from build123d import *

# Parameters (mm, degrees)
CENTER_BODY_SKETCH_W         = 80
CENTER_BODY_SKETCH_H         = 64
CENTER_BODY_SKETCH_R         = 17.5
CENTER_BODY_DEPTH            = 44
PIVOT_EYES_SKETCH_R          = 34
PIVOT_EYES_SKETCH_R_2        = 23.5
PIVOT_EYES_68X_47_DEPTH      = 15.75
PIVOT_EYES_68X_47_2_DEPTH    = 15.75
EYE_FACE_PADS_SKETCH_R       = 34
EYE_FACE_PADS_SKETCH_R_2     = 23.5
EYE_FACE_PADS_DEPTH          = 1.25
MOUNTING_LUG_A_SKETCH_W      = 27.466221721
MOUNTING_LUG_A_SKETCH_H      = 44
MOUNTING_LUG_A_SKETCH_R      = 4
MOUNTING_LUG_A_DEPTH         = 7
MOUNTING_START               = -14
MOUNTING_LUG_B_SKETCH_R      = 4
MOUNTING_LUG_B_DEPTH         = 14
OFFSET_PIVOT_EYES_SKETCH_R   = 34
OFFSET_PIVOT_EYES_SKETCH_R_2 = 23.5
OFFSET_PIVOT_EYES_DEPTH      = 8.5
CENTER_WEB_SKETCH_W          = 28.251394121
CENTER_WEB_SKETCH_H          = 44
CENTER_WEB_DEPTH             = 14
PIN_HOLE_SKETCH_R            = 3.5
PIN_HOLE_7_DEPTH             = 200
LUG_A_FILLETS_R5_R           = 5
LUG_B_FILLETS_R5_R           = 5


with BuildPart() as part:
    # Center Body Sketch → Center Body (new body)
    with BuildSketch(Plane(origin=(0, 0, 0), x_dir=(1, 0, 0), z_dir=(0, 1, 0))):
        Rectangle(CENTER_BODY_SKETCH_W, CENTER_BODY_SKETCH_H)
        with Locations(Location((0, 0, 0), (0, 0, 270))):
            Circle(CENTER_BODY_SKETCH_R, mode=Mode.SUBTRACT)
    extrude(amount=CENTER_BODY_DEPTH)



with BuildPart() as body_2:
    # Pivot Eyes Sketch → Pivot Eyes Ø68xØ47 (new body)
    with BuildSketch(Plane.XY.offset(32)):
        with Locations((-92.2, 22)):
            Circle(PIVOT_EYES_SKETCH_R)
        with Locations((-92.2, 22)):
            Circle(PIVOT_EYES_SKETCH_R_2, mode=Mode.SUBTRACT)
    extrude(amount=-PIVOT_EYES_68X_47_DEPTH)



with BuildPart() as body_3:
    # Pivot Eyes Sketch → Pivot Eyes _68x_47 2 (new body)
    with BuildSketch(Plane.XY.offset(32)):
        with Locations((92.2, 22)):
            Circle(PIVOT_EYES_SKETCH_R)
        with Locations((92.2, 22)):
            Circle(PIVOT_EYES_SKETCH_R_2, mode=Mode.SUBTRACT)
    extrude(amount=-PIVOT_EYES_68X_47_2_DEPTH)


with BuildPart() as body_2_1:
    add(body_2.part)

    add(body_3.part)  # Eye Face Pads merges body 3
    # Eye Face Pads Sketch → Eye Face Pads (add)
    # profile 1 of 2: a face of its own
    with BuildSketch(Plane.XY.offset(32)):
        with Locations((-92.2, 22)):
            Circle(EYE_FACE_PADS_SKETCH_R)
        with Locations((-92.2, 22)):
            Circle(EYE_FACE_PADS_SKETCH_R_2, mode=Mode.SUBTRACT)
    # profile 2 of 2: a face of its own
    with BuildSketch(Plane.XY.offset(32)):
        with Locations((92.2, 22)):
            Circle(EYE_FACE_PADS_SKETCH_R)
        with Locations((92.2, 22)):
            Circle(EYE_FACE_PADS_SKETCH_R_2, mode=Mode.SUBTRACT)
    extrude(amount=EYE_FACE_PADS_DEPTH)


with BuildPart() as part_1:
    add(part.part)

    add(body_2_1.part)  # Mounting Lug A merges body 2
    # Mounting Lug A Sketch → Mounting Lug A (add, symmetric)
    # profile 1 of 2: a face of its own
    with BuildSketch(Plane.XY.offset(25)):
        with Locations((53.733110861, 22)):
            Rectangle(MOUNTING_LUG_A_SKETCH_W, MOUNTING_LUG_A_SKETCH_H)
    # profile 2 of 2: a face of its own
    with BuildSketch(Plane.XY.offset(25)):
        with BuildLine():
            Line((-40, 44), (-40, 0))
            Line((-40, 0), (-66.277037206, 0))
            ThreePointArc((-66.277037206, 0), (-61.345502759, 36.282856857), (-92.2, 56))
            ThreePointArc((-92.2, 56), (-89.821719025, 56.601843613), (-88.015979336, 58.262488159))
            Line((-88.015979336, 58.262488159), (-73.833659926, 79.93878434))
            ThreePointArc((-73.833659926, 79.93878434), (-60.894229811, 86.47759422), (-48.760320341, 78.543293537))
            Line((-48.760320341, 78.543293537), (-32.680005104, 46.743691884))
            ThreePointArc((-32.680005104, 46.743691884), (-30.837059719, 44.740801685), (-28.218046601, 44))
            Line((-28.218046601, 44), (-40, 44))
        make_face()
        with Locations((-61.7, 72)):
            Circle(MOUNTING_LUG_A_SKETCH_R, mode=Mode.SUBTRACT)
    extrude(amount=MOUNTING_LUG_A_DEPTH, both=True)

    # Mounting Lug B Sketch → Mounting Lug B (add)
    with BuildSketch(Plane(origin=(0, 0, -32), x_dir=(-1, 0, 0), z_dir=(0, 0, -1)).offset(MOUNTING_START)):
        with BuildLine():
            Line((-40, 44), (-25.135268802, 44))
            ThreePointArc((-25.135268802, 44), (-27.59760019, 44.648342369), (-29.421358071, 46.425230346))
            Line((-29.421358071, 46.425230346), (-49.270341118, 79.466831997))
            ThreePointArc((-49.270341118, 79.466831997), (-61.764908832, 86.499854718), (-74.196010179, 79.355251839))
            Line((-74.196010179, 79.355251839), (-86.507393015, 58.439154252))
            ThreePointArc((-86.507393015, 58.439154252), (-88.41197553, 56.591508495), (-90.993751524, 55.978595683))
            ThreePointArc((-90.993751524, 55.978595683), (-61.096956424, 35.733196289), (-66.277037206, 0))
            Line((-66.277037206, 0), (-40, 0))
            Line((-40, 0), (-40, 44))
        make_face()
        with Locations((-61.7, 72)):
            Circle(MOUNTING_LUG_B_SKETCH_R, mode=Mode.SUBTRACT)
    extrude(amount=MOUNTING_LUG_B_DEPTH)

    # Offset Pivot Eyes Sketch → Offset Pivot Eyes (add, symmetric)
    # profile 1 of 2: a face of its own
    with BuildSketch(Plane.XY.offset(-25)):
        with Locations((92.2, 22)):
            Circle(OFFSET_PIVOT_EYES_SKETCH_R)
        with Locations((92.2, 22)):
            Circle(OFFSET_PIVOT_EYES_SKETCH_R_2, mode=Mode.SUBTRACT)
    # profile 2 of 2: a face of its own
    with BuildSketch(Plane.XY.offset(-25)):
        with Locations((-92.2, 22)):
            Circle(OFFSET_PIVOT_EYES_SKETCH_R)
        with Locations((-92.2, 22)):
            Circle(OFFSET_PIVOT_EYES_SKETCH_R_2, mode=Mode.SUBTRACT)
    extrude(amount=OFFSET_PIVOT_EYES_DEPTH, both=True)


with BuildPart() as offset_pivot_eyes_piece_1:
    # of the separate pieces the step leaves, piece 1, a body of its own (offset_pivot_eyes_pieces)
    add(part_1.part.solids().sort_by_distance((126.2, 22, -33.5))[0])



with BuildPart() as offset_pivot_eyes_piece_2:
    # of the separate pieces the step leaves, piece 2, a body of its own (offset_pivot_eyes_pieces)
    add(part_1.part.solids().sort_by_distance((-58.2, 22, -33.5))[0])


with BuildPart() as offset_pivot_eyes_piece_1_1:
    add(offset_pivot_eyes_piece_1.part)

    add(offset_pivot_eyes_piece_2.part)  # Center Web merges Offset Pivot Eyes piece 2
    # Center Web Sketch → Center Web (add)
    with BuildSketch(Plane(origin=(0, 0, -32), x_dir=(-1, 0, 0), z_dir=(0, 0, -1))):
        with Locations((54.125697061, 22)):
            Rectangle(CENTER_WEB_SKETCH_W, CENTER_WEB_SKETCH_H)
    extrude(amount=-CENTER_WEB_DEPTH)

    # Pin Hole Sketch → Pin Hole Ø7 (cut)
    with BuildSketch(Plane(origin=(0, 0, -32), x_dir=(-1, 0, 0), z_dir=(0, 0, -1))):
        with Locations((0, 22)):
            Circle(PIN_HOLE_SKETCH_R)
    extrude(amount=-PIN_HOLE_7_DEPTH, mode=Mode.SUBTRACT)

    # Lug A Fillets R5
    lug_a_fillets_r5_edges = [offset_pivot_eyes_piece_1_1.edges().sort_by_distance(p)[0] for p in [
        (-40, 22, -18),
        (-40, 22, 18),
    ]]
    fillet(lug_a_fillets_r5_edges, radius=LUG_A_FILLETS_R5_R)

    # Lug B Fillets R5
    lug_b_fillets_r5_edges = [offset_pivot_eyes_piece_1_1.edges().sort_by_distance(p)[0] for p in [
        (40, 22, 18),
        (40, 22, -18),
    ]]
    fillet(lug_b_fillets_r5_edges, radius=LUG_B_FILLETS_R5_R)


solid = offset_pivot_eyes_piece_1_1.part
Design review of the part built by this model. Coordinates are the model's own, in mm. A direction names the side the tool comes from. Round coordinates to 2 decimals unless told otherwise and drop trailing zeros. Write each loop counter-clockwise with the first axis right and the second up, starting at its lowest first coordinate (ties: lowest second). Pieces come first, ordered by that corner, then holes. Notation, with made-up numbers: M -38,-30.5 L -13,-30.5 A18 cw -13,-16.5 Z; hole C 74,52 d11. An arc over 180 degrees is marked long. One line per item, written item: value. Start each with the question number.
1. Clearance check with flat-ended pins moving along their axes: P1, Ø1, axis at x = 30, y = 16, coming from the +Z side; P2, Ø6, axis at y = 8.5, z = 5.5, coming from the +X side; P3, Ø3, axis at x = -50, z = 22.5, coming from the +Y side. State where each tip first meets the part, or that it passes through.
2. Take a section at B-B on z = 24. State the section outline as (x, y) points.
3. Take a section at C-C on y = 61.5. State the section outline as (x, z) points, then the cut area to 3 significant figures.
4. Take a section at D-D on z = 0. State the section outline as (x, y) points.
5. Draft analysis for pull direction Z (two halves, no side actions). For faces 6 (the face through (5.26, 21.69, 16.69)), 7 (the face through (27.566, 44.631, -24.902)), 8 (the face through (-115, 15, -33.5)), state which applies: pulls with the +Z half, pulls with the -Z half, needs draft (parallel to the pull), parting line crosses it, or undercut.
6. Take a section at A-A on x = 0. State the section outline as (y, z) points.
7. To check wall thickness, follow probe 1 along Y at (x, z) = (0, -25.75); probe 2 along Y at (x, z) = (-92, -22); probe 3 along Z at (x, y) = (0, 16). State the ranges of each line that lie inside material, in increasing order. Write a range as from..to.
8. For faces 1 (the face through (-81.024, 68.949, 25.098)), 2 (the face through (-41, 22, -16)), 3 (the face through (64.9, 69.6, -24.9)), 4 (the face through (69, 15, 16.25)), 5 (the face through (-115, 15, 16.25)), list the 3-axis set-ups (+Z, -Z, +X, -X, +Y, -Y) from which the entire face can be reached by the end or side of a thin tool; tool diameter is ignored.
Computed:
1. P1: stops at z = 32
1. P2: stops at x = 40
1. P3: stops at y = 82.31
2. outline: M -92.2,56 A34 ccw long -66.28,0 L 66.28,0 A34 ccw long 66.28,44 L -28.22,44 A5 cw -32.68,46.74 L -48.76,78.54 A14.5 ccw -73.83,79.94 L -88.02,58.26 A5 cw Z; hole C -92.2,22 d47; hole C -61.7,72 d8; hole C 0,22 d7; hole C 92.2,22 d47
3. outline: M -85.9,18 L -40.14,18 L -40.14,32 L -85.9,32 Z; M 38.48,-32 L 84.71,-32 L 84.71,-18 L 38.48,-18 Z
3. area: 1,290 mm²
4. outline: M -40,0 L -17.5,0 L -17.5,44 L -40,44 Z; M 17.5,0 L 40,0 L 40,44 L 17.5,44 Z
5. face 6: undercut
5. face 7: needs draft
5. face 8: pulls with the -Z half
6. outline: M 0,-32 L 18.5,-32 L 18.5,-17.5 L 0,-17.5 Z; M 0,17.5 L 18.5,17.5 L 18.5,32 L 0,32 Z; M 25.5,-32 L 44,-32 L 44,-17.5 L 25.5,-17.5 Z; M 25.5,17.5 L 44,17.5 L 44,32 L 25.5,32 Z
7. probe 1: y = 0..18.5, 25.5..44
7. probe 2: y = -12..-1.5, 45.5..56
7. probe 3: z = -32..-17.5, 17.5..32
8. face 1: +Z, -Z, -X, +Y
8. face 2: +Y, -Y
8. face 3: +Z, -Z
8. face 4: +X, +Y, -Y
8. face 5: -X, +Y, -Y
